The drawing under review shows one solid part. Ordinate dimensions are in mm from its lowest x, y, z. A direction names the side the tool comes from. Coordinates: 2 decimals unless noted, no trailing zeros. Loops run counter-clockwise (first coordinate to the right, second up) from the corner with the lowest first, then second, coordinate; pieces in that order, holes last. Notation, with made-up numbers: M -11.75,27 L 2.25,27 A25 ccw 2.25,47 Z; hole C 23,-19 d1. An arc over 180 degrees is marked long. Answer as a JSON object with one key per item and string values. Group by question number.
1. Consider section C-C (x = 5.5). State the section outline as (y, z) points (1 decimal).
2. Machinability: for the marked faces 1, 2 and 3, which of the approach directions +Z, -Z, +X, -X, +Y, -Y give a long, thin tool a straight path to every point of the face, cutting with its end or side? Answer none if there is none.
3. To check wall thickness, follow probe 1 along Y at (x, z) = (61, 3.5); probe 2 along Y at (x, z) = (5, 2.75); probe 3 along X at (y, z) = (8.25, 6.25) (1 decimal). State the ranges of each line that lie inside material, in increasing order.
4. Consider section A-A (y = 7.5). State the section outline as (x, z) points.
5. Insertion check: pin 1 (1.2 mm diameter, centred on x = 32, z = 4, fed in from -Y); pin 2 (4 mm diameter, centred on y = 5, z = 7, fed in from +X); pin 3 (2 mm diameter, centred on x = 42.5, z = 5.5, fed in from +Y); pin 4 (4 mm diameter, centred on x = 56.5, y = 11, fed in from -Z). Each pin has a flat end and moves straight along its axis. Give the tip position at first contact, or say it passes through.
6. Consider section B-B (z = 7). State the section outline as (x, y) points.
7. Consider section D-D (z = 3.75). State the section outline as (x, y) points (1 decimal).
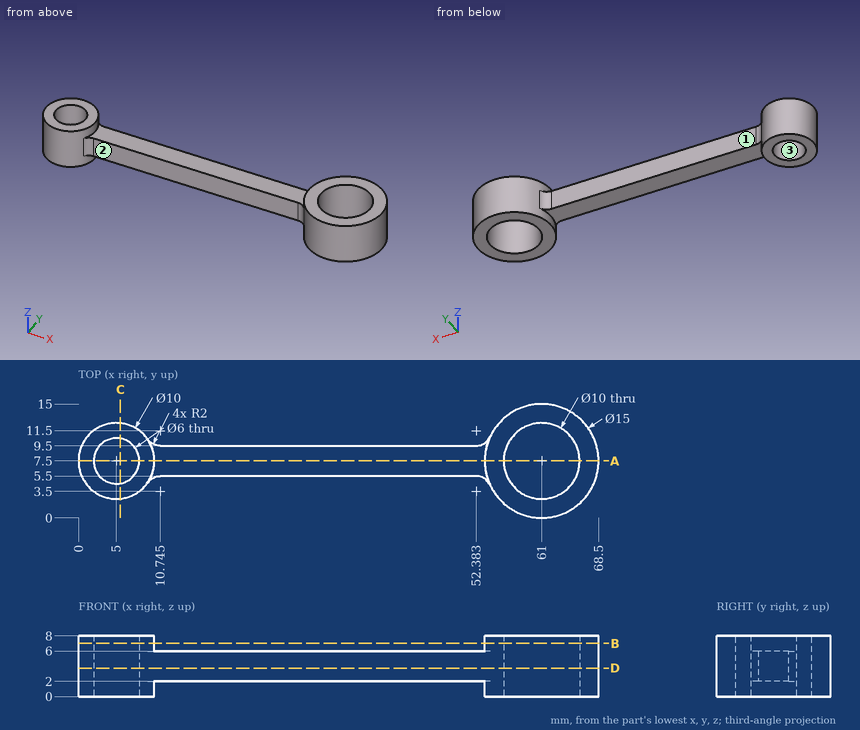
Findings below:
{
 "1": {"outline": "M 2.5,0 L 4.5,0 L 4.5,8 L 2.5,8 Z; M 10.5,0 L 12.5,0 L 12.5,8 L 10.5,8 Z"},
 "2": {"face 1": "+Z, -Z, +Y", "face 2": "+Z, -Z, -Y", "face 3": "+Z, -Z"},
 "3": {"probe 1": "y = 0 to 2.5, 12.5 to 15", "probe 2": "y = 2.5 to 4.5, 10.5 to 12.5", "probe 3": "x = 0.1 to 2.1, 7.9 to 9.9, 53.5 to 56.1, 65.9 to 68.5"},
 "4": {"outline": "M 0,0 L 2,0 L 2,8 L 0,8 Z; M 8,0 L 10,0 L 10,2 L 53.5,2 L 53.5,0 L 56,0 L 56,8 L 53.5,8 L 53.5,6 L 10,6 L 10,8 L 8,8 Z; M 66,0 L 68.5,0 L 68.5,8 L 66,8 Z"},
 "5": {"pin 1": "stops at y = 5.5", "pin 2": "stops at x = 68.48", "pin 3": "stops at y = 9.5", "pin 4": "stops at z = 0"},
 "6": {"outline": "C 5,7.5 d10; C 61,7.5 d15; hole C 5,7.5 d6; hole C 61,7.5 d10"},
 "7": {"outline": "M 9.1,4.6 A2 cw 10.7,5.5 L 52.4,5.5 A2 cw 54.2,4.3 A7.5 ccw long 54.2,10.7 A2 cw 52.4,9.5 L 10.7,9.5 A2 cw 9.1,10.4 A5 ccw long Z; hole C 5,7.5 d6; hole C 61,7.5 d10"}
}
